```python
from build123d import *

# Parameters (mm, degrees)
EXTRUDE_1_DEPTH          = 35
CUT_EXTRUDE_1_DEPTH      = 1448.428754723
CUT_EXTRUDE_1_DEPTH_BACK = 1448.428754723
CHAMFER_2_SIZE           = 20
CUT_EXTRUDE_2_DEPTH      = 1448.428754723
CUT_EXTRUDE_2_DEPTH_BACK = 1448.428754723
SKETCH_5_R               = 11


with BuildPart() as part:
    # 草图1 → 凸台-拉伸1 (new body)
    with BuildSketch(Plane(origin=(0, 0, 0), x_dir=(1, 0, 0), z_dir=(0, 1, 0))):
        Polygon((-1160, 500), (-810, 500), (-810, 865), (-710, 865), (-710, 745), (-230, 745), (-230, 865), (-130, 865), (-130, 500), (0, 500), (0, 0), (-1160, 0), align=None)
    extrude(amount=EXTRUDE_1_DEPTH)

    # 草图4 → 切除-拉伸1 (cut, two sides: drawn at the far end of the back side and taken through both)
    with BuildSketch(Plane(origin=(0, 35, 0), x_dir=(1, 0, 0), z_dir=(0, 1, 0)).offset(-CUT_EXTRUDE_1_DEPTH_BACK)):
        Polygon((-230, 745), (-710, 745), (-710, 380), (-1040, 380), (-1040, 120), (-120, 120), (-120, 380), (-230, 380), align=None)
    extrude(amount=CUT_EXTRUDE_1_DEPTH + CUT_EXTRUDE_1_DEPTH_BACK, mode=Mode.SUBTRACT)

    # 倒角2
    chamfer_2_edges = [part.edges().sort_by_distance(p)[0] for p in [
        (0, 17.5, 0),
        (-1160, 17.5, 0),
        (-1160, 17.5, -500),
        (-810, 17.5, -865),
        (-130, 17.5, -865),
        (0, 17.5, -500),
    ]]
    chamfer(chamfer_2_edges, length=CHAMFER_2_SIZE)

    # 草图5 → 切除-拉伸2 (cut, two sides: drawn at the far end of the back side and taken through both)
    with BuildSketch(Plane(origin=(0, 35, 0), x_dir=(1, 0, 0), z_dir=(0, 1, 0)).offset(-CUT_EXTRUDE_2_DEPTH_BACK)):
        with Locations(Location((-1120, 40, 0), (0, 0, 270))):
            Circle(SKETCH_5_R)
        with Locations(Location((-970, 40, 0), (0, 0, 270))):
            Circle(SKETCH_5_R)
        with Locations(Location((-820, 40, 0), (0, 0, 270))):
            Circle(SKETCH_5_R)
        with Locations(Location((-670, 40, 0), (0, 0, 270))):
            Circle(SKETCH_5_R)
        with Locations(Location((-490, 40, 0), (0, 0, 270))):
            Circle(SKETCH_5_R)
        with Locations(Location((-340, 40, 0), (0, 0, 270))):
            Circle(SKETCH_5_R)
        with Locations(Location((-190, 40, 0), (0, 0, 270))):
            Circle(SKETCH_5_R)
        with Locations(Location((-40, 40, 0), (0, 0, 270))):
            Circle(SKETCH_5_R)
        with Locations(Location((-770, 825, 0), (0, 0, 270))):
            Circle(SKETCH_5_R)
        with Locations(Location((-770, 695, 0), (0, 0, 270))):
            Circle(SKETCH_5_R)
        with Locations(Location((-770, 565, 0), (0, 0, 270))):
            Circle(SKETCH_5_R)
        with Locations(Location((-770, 460, 0), (0, 0, 270))):
            Circle(SKETCH_5_R)
        with Locations(Location((-1120, 180, 0), (0, 0, 270))):
            Circle(SKETCH_5_R)
        with Locations(Location((-1120, 250, 0), (0, 0, 270))):
            Circle(SKETCH_5_R)
        with Locations(Location((-1120, 320, 0), (0, 0, 270))):
            Circle(SKETCH_5_R)
        with Locations(Location((-1120, 460, 0), (0, 0, 270))):
            Circle(SKETCH_5_R)
        with Locations(Location((-950, 460, 0), (0, 0, 270))):
            Circle(SKETCH_5_R)
        with Locations(Location((-170, 460, 0), (0, 0, 90))):
            Circle(SKETCH_5_R)
        with Locations(Location((-170, 565, 0), (0, 0, 90))):
            Circle(SKETCH_5_R)
        with Locations(Location((-170, 695, 0), (0, 0, 90))):
            Circle(SKETCH_5_R)
        with Locations(Location((-170, 825, 0), (0, 0, 90))):
            Circle(SKETCH_5_R)
        with Locations(Location((-40, 460, 0), (0, 0, 270))):
            Circle(SKETCH_5_R)
        with Locations(Location((-40, 320, 0), (0, 0, 270))):
            Circle(SKETCH_5_R)
        with Locations(Location((-40, 180, 0), (0, 0, 270))):
            Circle(SKETCH_5_R)
    extrude(amount=CUT_EXTRUDE_2_DEPTH + CUT_EXTRUDE_2_DEPTH_BACK, mode=Mode.SUBTRACT)


solid = part.part
```
The listing builds one solid part. Answer for the finished solid, in the listing's coordinates (mm). A direction names the side the tool comes from. Round coordinates to 2 decimals unless told otherwise and drop trailing zeros. Loops run counter-clockwise (first coordinate to the right, second up) from the corner with the lowest first, then second, coordinate; pieces in that order, holes last. Notation, with made-up numbers: (-4.5, 37) - (25.5, 37) arc R5 cw to (25.5, 46) - close; hole circle Ø2 at (45.5, 9). An arc over 180 degrees is marked (long way). Return JSON: item names as keys, results as strings. Group by question number.
1. Consider probe 1 along Z at (x, y) = (-190, 19); probe 2 along X at (y, z) = (25, -320); probe 3 along X at (y, z) = (9.5, -356). Determine where each line is inside the solid, lowest interval first.
2. The part is cut by section A-A on z = -661.5. Determine the outline of the cut face in (x, y).
3. The part is cut by section C-C on y = 18. State how many separate pieces and enclosed holes the cut face has, then the cut area to 3 significant figures.
4. The mould has two halves that part along X. Classify faces 4 (the flat face through (0, 17, -253)), 5 (the flat face through (-751, 17, -865)), 6 (the cylindrical face through (-40, 17, -331)), 7 (the flat face through (-810, 17, -670)): pulls with the +X half, pulls with the -X half, needs draft (parallel to the pull), parting line crosses it, or undercut.
5. Each of these flat-tipped pins is pushed along its axis until it touches: P1, Ø8, axis at y = 12.5, z = -775, coming from the -X side; P2, Ø2, axis at y = 5, z = -608, coming from the +X side; P3, Ø10.5, axis at x = -51.5, y = 13.5, coming from the -Z side. Where does it stop, or does it pass through?
6. The part is cut by section B-B on x = -874. Determine the outline of the cut face in (y, z).
7. The part is cut by section D-D on x = -462. Determine the outline of the cut face in (y, z), then the cut area to 3 significant figures.
8. Which of the six approach directions +Z, -Z, +X, -X, +Y, -Y give full straight-line access (tool end or side, diameter ignored) to faces 1 (the flat face through (-572, 17, 0)), 2 (the flat face through (-873, 17, -380)), 3 (the flat face through (-130, 17, -675))?
Resolved:
{
 "1": {"probe 1": "z = -865 to -380, -120 to -51, -29 to 0", "probe 2": "x = -1160 to -1131, -1109 to -1040, -120 to -51, -29 to 0", "probe 3": "x = -1160 to -1040, -120 to 0"},
 "2": {"outline": "(-810, 0) - (-710, 0) - (-710, 35) - (-810, 35) - close; (-230, 0) - (-130, 0) - (-130, 35) - (-230, 35) - close"},
 "3": {"separate pieces": "1", "enclosed holes": "24", "area": "346,000 mm²"},
 "4": {"face 4": "pulls with the +X half", "face 5": "needs draft", "face 6": "undercut", "face 7": "pulls with the -X half"},
 "5": {"P1": "stops at x = -810", "P2": "stops at x = -130", "P3": "stops at z = -500"},
 "6": {"outline": "(0, -500) - (35, -500) - (35, -380) - (0, -380) - close; (0, -120) - (35, -120) - (35, 0) - (0, 0) - close"},
 "7": {"outline": "(0, -120) - (35, -120) - (35, 0) - (0, 0) - close", "area": "4,200 mm²"},
 "8": {"face 1": "+Z, +X, -X, +Y, -Y", "face 2": "+Y, -Y", "face 3": "-Z, +X, +Y, -Y"}
}
